Build history of the part. All positions in model axes, mm. Round coordinates to 2 decimals unless told otherwise and drop trailing zeros. Loops run counter-clockwise (first coordinate to the right, second up) from the corner with the lowest first, then second, coordinate; pieces in that order, holes last. Notation, with made-up numbers: M -28,10 L -16,10 A24 cw -16,40 Z; hole C 16,-4.5 d10. An arc over 180 degrees is marked long. Use one line per item in the form item = value. Start each with the question number.
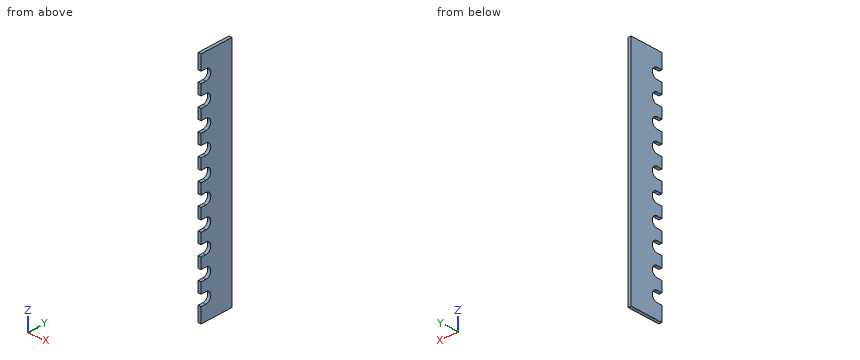
```python
from build123d import *

# Parameters (mm, degrees)
SKETCH1_W           = 3
SKETCH1_H           = 32
EXTRUDE_THIN1_DEPTH = 218
CUT_EXTRUDE1_DEPTH  = 221.356529288
LPATTERN1_COUNT     = 10
LPATTERN1_PITCH     = 20


with BuildPart() as part:
    # Sketch1 → Extrude-Thin1 (new body)
    with BuildSketch(Plane.XY):
        with Locations((-1.5, -16)):
            Rectangle(SKETCH1_W, SKETCH1_H)
    extrude(amount=EXTRUDE_THIN1_DEPTH)

    # Sketch2 → Cut-Extrude1 (cut, through all)
    with BuildSketch(Plane(origin=(0, 0, 0), x_dir=(0, 0, -1), z_dir=(1, 0, 0))):
        with BuildLine():
            Line((-194, -27), (-194, -32))
            Line((-194, -32), (-204, -32))
            Line((-204, -32), (-204, -27))
            ThreePointArc((-204, -27), (-199, -22), (-194, -27))
        make_face()
    cut_extrude1 = extrude(amount=-CUT_EXTRUDE1_DEPTH, mode=Mode.SUBTRACT)

    # LPattern1: Cut-Extrude1 ×10
    with Locations(*[(0, 0, -i * LPATTERN1_PITCH) for i in range(1, LPATTERN1_COUNT)]):
        add(cut_extrude1, mode=Mode.SUBTRACT)


solid = part.part
```
Q1. Saw through at A-A (y = -29). Give the number of separate pieces and of enclosed holes in the cut face, and give its area (3 significant figures).
Q2. Saw through at C-C (z = 97). Give the cut face in (x, y).
Q3. Saw through at B-B (z = 179). Give the cut face in (x, y), and give its area (3 significant figures).
Q4. Wall check: probe 1 along Y at (x, z) = (-2.2, 178); probe 2 along Y at (x, z) = (-0.95, 176). Give the ranges that are in metal, low to high.
Filled in:
q1.separate_pieces = 11
q1.enclosed_holes = 0
q1.area = 354 mm²
q2.outline = M -3,-22.42 L 0,-22.42 L 0,0 L -3,0 Z
q3.outline = M -3,-22 L 0,-22 L 0,0 L -3,0 Z
q3.area = 66.0 mm²
q4.probe_1 = -22.1 to 0
q4.probe_2 = -23 to 0
